The listing builds one solid part. Answer for the finished solid, in the listing's coordinates (mm). Face numbers are marked on the shaded views. A direction names the side the tool comes from. Coordinates: 2 decimals unless noted, no trailing zeros. Loops run counter-clockwise (first coordinate to the right, second up) from the corner with the lowest first, then second, coordinate; pieces in that order, holes last. Notation, with made-up numbers: M 48,11 L 92,11 A21 cw 92,15 Z; hole C -17.5,-11.75 d4. An arc over 180 degrees is marked long. Return JSON: item names as keys, results as strings. Group by question number.
1. Section B-B (y = 5.5) is taken. Write down the section's boundary in (x, z), then the cut area to 3 significant figures.
2. Straight lines are drawn through the part: L1, parallel to Y at x = 0, z = 11; L2, parallel to Z at x = -2.75, y = 48; L3, parallel to Y at x = 2.75, z = 6.25. For each, find the intervals that lie inside material, in ascending order. Write a range as from..to.
3. Which of the six approach directions +Z, -Z, +X, -X, +Y, -Y give full straight-line access (tool end or side, diameter ignored) to the marked faces 1, 2 and 3?
4. Section D-D (x = 4.25) is taken. Write down the section's boundary in (y, z), then the cut area to 3 significant figures.
5. The mould has two halves that part along X. Classify the marked faces 4, 5, 6 and 7: pulls with the +X half, pulls with the -X half, needs draft (parallel to the pull), parting line crosses it, or undercut.
6. Given P1, Ø3, axis at x = -2.5, y = 42.5, coming from the -Z side; P2, Ø1.8, axis at x = -1.5, z = 6, coming from the -Y side; P3, Ø3, axis at x = 0, y = 0, coming from the -Z side; P4, Ø2, axis at x = -2.5, z = 9.5, coming from the -Y side, each flat-ended and moving along its own axis, determine where each tip first touches the part or whether it passes through.
7. Section A-A (x = 0) is taken. Count the separate pieces of the cut face and the enclosed holes in it, then the cut area to 3 significant figures.
8. Section C-C (z = 4.5) is taken. Write down the section's boundary in (x, y), then the cut area to 3 significant figures.
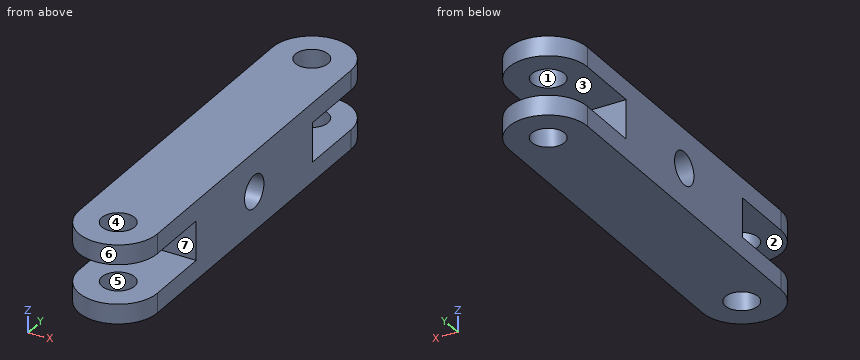
```python
from build123d import *

# Parameters (mm, degrees)
BOSS_EXTRUDE1_DEPTH = 12
SKETCH2_W           = 6
SKETCH2_H           = 32
CUT_EXTRUDE1_DEPTH  = 59.514955353
SKETCH3_R           = 2.5
CUT_EXTRUDE2_DEPTH  = 58.584720196
M6_TAPPED_HOLE1_D   = 5


with BuildPart() as part:
    # Sketch1 → Boss-Extrude1 (new body)
    with BuildSketch(Plane.XY):
        with BuildLine():
            Line((-6, 0), (-6, 50))
            ThreePointArc((-6, 50), (0, 56), (6, 50))
            Line((6, 50), (6, 0))
            ThreePointArc((6, 0), (0, -6), (-6, 0))
        make_face()
    extrude(amount=BOSS_EXTRUDE1_DEPTH)

    # Sketch2 → Cut-Extrude1 (cut, through all)
    with BuildSketch(Plane.ZY.offset(6)):
        with Locations((6, 56)):
            Rectangle(SKETCH2_W, SKETCH2_H)
        with Locations((6, -6)):
            Rectangle(SKETCH2_W, SKETCH2_H)
    extrude(amount=-CUT_EXTRUDE1_DEPTH, mode=Mode.SUBTRACT)

    # Sketch3 → Cut-Extrude2 (cut, through all)
    with BuildSketch(Plane.XY.offset(12)):
        with Locations((0, 50)):
            Circle(SKETCH3_R)
        Circle(SKETCH3_R)
    extrude(amount=-CUT_EXTRUDE2_DEPTH, mode=Mode.SUBTRACT)

    # M6 Tapped Hole1 (through all)
    with Locations(Plane(origin=(6, 25, 6), x_dir=(0, 0, 1), z_dir=(1, 0, 0))):
        with Locations((0, 0)):
            Hole(M6_TAPPED_HOLE1_D / 2)


solid = part.part
```
Worked out:
{
 "1": {"outline": "M -6,0 L 6,0 L 6,3 L -6,3 Z; M -6,9 L 6,9 L 6,12 L -6,12 Z", "area": "72.0 mm^2"},
 "2": {"L1": "-6..-2.5, 2.5..47.5, 52.5..56", "L2": "0..3, 9..12", "L3": "10..22.51, 27.49..40"},
 "3": {"face 1": "+Z, -Z", "face 2": "+X, -X, -Y", "face 3": "+X, -X, +Y"},
 "4": {"outline": "M -4.24,0 L 54.24,0 L 54.24,3 L 40,3 L 40,9 L 54.24,9 L 54.24,12 L -4.24,12 L -4.24,9 L 10,9 L 10,3 L -4.24,3 Z; hole C 25,6 d5", "area": "511 mm^2"},
 "5": {"face 4": "undercut", "face 5": "undercut", "face 6": "parting line crosses it", "face 7": "needs draft"},
 "6": {"P1": "z = 0", "P2": "y = 10", "P3": "through", "P4": "y = -5.81"},
 "7": {"separate pieces": "5", "enclosed holes": "1", "area": "472 mm^2"},
 "8": {"outline": "M -6,10 L 6,10 L 6,23 L -6,23 Z; M -6,27 L 6,27 L 6,40 L -6,40 Z", "area": "312 mm^2"}
}
